Build history of the part. All positions in model axes, mm. A direction names the side the tool comes from. Give positions to 0.01 mm unless a question says otherwise; leave off trailing zeros. Order: outer loops, then holes, each group sorted by start corner. A loop starts at its lowest first (then second) coordinate and runs counter-clockwise, first axis right, second up. Notation, with made-up numbers: (71, 55) -> (104, 55) arc R19 cw to (104, 86) -> close; hole circle Ø1 at (15.25, 16). An arc over 180 degrees is marked (long way). Use a Markdown table: item, result. Add a question column.
```python
from build123d import *

# Parameters (mm, degrees)
EXTRUDE_1_DEPTH     = 6
SKETCH_2_W          = 64
SKETCH_2_H          = 50
CUT_EXTRUDE_1_DEPTH = 2


with BuildPart() as part:
    # 草图1 → 凸台-拉伸1 (new, symmetric)
    with BuildSketch(Plane.XY):
        Polygon((0, 0), (0, 60), (-14, 60), (-59, 105), (-239, 105), (-239, 155), (30, 155), (30, 0), align=None)
    extrude(amount=EXTRUDE_1_DEPTH, both=True)

    # 草图2 → 切除-拉伸1 (cut)
    with BuildSketch(Plane(origin=(0, 0, 6), x_dir=(-1, 0, 0), z_dir=(0, 0, -1))):
        with Locations((187, 130)):
            Rectangle(SKETCH_2_W, SKETCH_2_H)
    extrude(amount=CUT_EXTRUDE_1_DEPTH, mode=Mode.SUBTRACT)


solid = part.part
```
(1) Band-saw the part on A-A on y = 119.5. Give the cut face in (x, z), plus the area to 3 significant figures.
(2) Band-saw the part on B-B on z = -0.5. Give the cut face in (x, y), plus the area to 3 significant figures.
(3) Mould opens along X. For faces 1 (the face through (-36, 82, 0)), 2 (the face through (30, 79, 0)), 3 (the face through (15, 0, 0)), 4 (the face through (-187, 130, 4)) say: released by +X, released by -X, zero draft, split by the parting line, or undercut.
(4) Pin check, flat tips, straight feed: pin 1 Ø3.5 at (x, z) = (-4, 2) entering from -Y; pin 2 Ø25 at (x, y) = (-182.5, 139) entering from +Z. Stop position of each tip, or through.
(5) Band-saw the part on D-D on y = 87. Give the cut face in (x, z), plus the area to 3 significant figures.
(6) Tool access for faces 5 (the face through (0, 30, 0)), 6 (the face through (-41, 113, 6)): list every direction of +Z, -Z, +X, -X, +Y, -Y with a clear straight run to the whole face (end or side of a thin tool).
(7) Band-saw the part on C-C on x = -134. Give the cut face in (y, z), plus the area to 3 significant figures.
(8) Wall check: probe 1 along X at (y, z) = (44, -3.75); probe 2 along Y at (x, z) = (-163, -4); probe 3 along Y at (x, z) = (-12.5, 5.25). Give the ranges that are in metal, low to high.
Response:
| question | item | result |
|---|---|---|
| 1 | outline | (-239, -6) -> (30, -6) -> (30, 6) -> (-155, 6) -> (-155, 4) -> (-219, 4) -> (-219, 6) -> (-239, 6) -> close |
| 1 | area | 3,100 mm² |
| 2 | outline | (-239, 105) -> (-59, 105) -> (-14, 60) -> (0, 60) -> (0, 0) -> (30, 0) -> (30, 155) -> (-239, 155) -> close |
| 2 | area | 18,200 mm² |
| 3 | face 1 | released by -X |
| 3 | face 2 | released by +X |
| 3 | face 3 | zero draft |
| 3 | face 4 | undercut |
| 4 | pin 1 | stops at y = 60 |
| 4 | pin 2 | stops at z = 4 |
| 5 | outline | (-41, -6) -> (30, -6) -> (30, 6) -> (-41, 6) -> close |
| 5 | area | 852 mm² |
| 6 | face 5 | +Z, -Z, -X, -Y |
| 6 | face 6 | +Z, +X, -X, +Y, -Y |
| 7 | outline | (105, -6) -> (155, -6) -> (155, 6) -> (105, 6) -> close |
| 7 | area | 600 mm² |
| 8 | probe 1 | x = 0 to 30 |
| 8 | probe 2 | y = 105 to 155 |
| 8 | probe 3 | y = 60 to 155 |
